Read the model definition and answer for the solid it produces. Units are mm, in the model's axes. Face numbers are marked on the shaded views. A direction names the side the tool comes from. Coordinates: 2 decimals unless noted, no trailing zeros. Write each loop counter-clockwise with the first axis right and the second up, starting at its lowest first coordinate (ties: lowest second). Pieces come first, ordered by that corner, then holes.
(1) Given pin 1 (1 mm diameter, centred on y = -12.5, z = 103.5, fed in from -X); pin 2 (6 mm diameter, centred on y = -16.5, z = 56.5, fed in from -X); pin 3 (8 mm diameter, centred on x = -8.5, z = 9.5, fed in from +Y), each flat-ended and moving along its own axis, determine where each tip first touches the part or whether it passes through.
(2) The part is cut by section A-A, the plane y = 0. Determine the outline of the cut face in (x, z), and give its area (3 significant figures).
(3) Straight lines are drawn through the part: line 1 along X through (y, z) = (-1, 68.5); line 2 along X through (y, z) = (-1, 105); line 3 along Z through (x, y) = (21.5, 11.5). For each, find the intervals that lie inside material, in ascending order.
(4) The part is cut by section D-D, the plane z = -103. Determine the outline of the cut face in (x, y).
(5) The part is cut by section C-C, the plane z = 21. Determine the outline of the cut face in (x, y), and give its area (3 significant figures).
(6) Which of the six approach directions +Z, -Z, +X, -X, +Y, -Y give full straight-line access (tool end or side, diameter ignored) to the marked faces 1, 2 and 3?
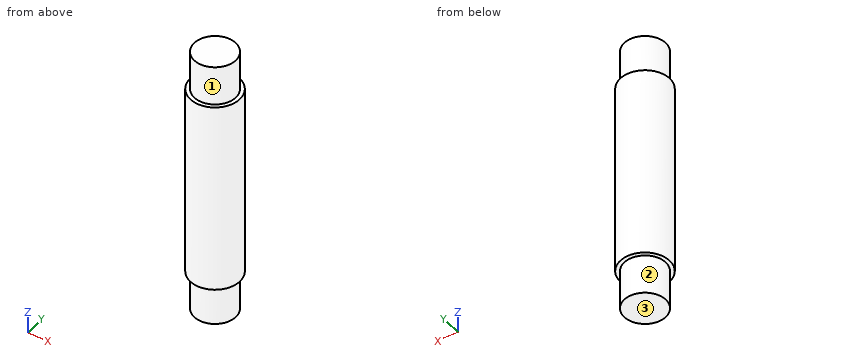
```python
from build123d import *

# Parameters (mm, degrees)
SKETCH_1_R           = 25
BOSS_EXTRUDE_1_DEPTH = 98
SKETCH_2_R           = 21
BOSS_EXTRUDE_2_DEPTH = 40


with BuildPart() as part:
    # Sketch 1 → Boss-Extrude 1 (new, symmetric)
    with BuildSketch(Plane.XY):
        Circle(SKETCH_1_R)
    extrude(amount=BOSS_EXTRUDE_1_DEPTH, both=True)

    # Sketch 2 → Boss-Extrude 2 (add)
    with BuildSketch(Plane.XY.offset(98)):
        Circle(SKETCH_2_R)
    boss_extrude_2 = extrude(amount=BOSS_EXTRUDE_2_DEPTH)

    # Mirror 1: Boss-Extrude 2 across plane
    add(boss_extrude_2.mirror(Plane.XY))


solid = part.part
```
Computed:
1. pin 1: stops at x = -17.23
1. pin 2: stops at x = -21.04
1. pin 3: stops at y = 24.59
2. outline: (-25, -98) - (-21, -98) - (-21, -138) - (21, -138) - (21, -98) - (25, -98) - (25, 98) - (21, 98) - (21, 138) - (-21, 138) - (-21, 98) - (-25, 98) - close
2. area: 13,200 mm2
3. line 1: x = -24.98 to 24.98
3. line 2: x = -20.98 to 20.98
3. line 3: z = -98 to 98
4. outline: circle Ø42 at (0, 0)
5. outline: circle Ø50 at (0, 0)
5. area: 1,960 mm2
6. face 1: +Z
6. face 2: -Z
6. face 3: -Z, +X, -X, +Y, -Y
